from build123d import *

# Parameters (mm, degrees)
SKETCH1_W             = 220
SKETCH1_H             = 90
BOSS_EXTRUDE1_DEPTH   = 15
M6_TAPPED_HOLE1_D     = 5
M6_TAPPED_HOLE1_DEPTH = 15
M6_TAPPED_HOLE1_TIP   = 1.502151548
CUT_EXTRUDE1_DEPTH    = 239.170107276
CUT_EXTRUDE2_DEPTH    = 239.170107276
M6_TAPPED_HOLE2_D     = 5
M6_TAPPED_HOLE2_DEPTH = 15
M6_TAPPED_HOLE2_TIP   = 1.502151548
CHAMFER1_SIZE         = 5
FILLET1_R             = 5
CUT_EXTRUDE3_DEPTH    = 6
SKETCH11_R            = 2.5
CUT_EXTRUDE4_DEPTH    = 239.170107276


with BuildPart() as part:
    # Sketch1 → Boss-Extrude1 (new body)
    with BuildSketch(Plane.XY):
        with Locations((110, 45)):
            Rectangle(SKETCH1_W, SKETCH1_H)
    extrude(amount=BOSS_EXTRUDE1_DEPTH)

    # M6 Tapped Hole1
    with Locations(Plane.XY.offset(15)):
        with Locations((70, 73), (70, 17), (200, 73), (200, 17)):
            Hole(M6_TAPPED_HOLE1_D / 2, depth=M6_TAPPED_HOLE1_DEPTH)
            with Locations((0, 0, -(M6_TAPPED_HOLE1_DEPTH + M6_TAPPED_HOLE1_TIP / 2))):  # 118° drill point
                Cone(0, M6_TAPPED_HOLE1_D / 2, M6_TAPPED_HOLE1_TIP, mode=Mode.SUBTRACT)

    # Sketch4 → Cut-Extrude1 (cut, through all)
    with BuildSketch(Plane.XY.offset(15)):
        with BuildLine():
            Line((44.5, 80), (44.5, 70))
            ThreePointArc((44.5, 70), (40, 65.5), (35.5, 70))
            Line((35.5, 70), (35.5, 80))
            ThreePointArc((35.5, 80), (40, 84.5), (44.5, 80))
        make_face()
        with BuildLine():
            Line((44.5, 20), (44.5, 10))
            ThreePointArc((44.5, 10), (40, 5.5), (35.5, 10))
            Line((35.5, 10), (35.5, 20))
            ThreePointArc((35.5, 20), (40, 24.5), (44.5, 20))
        make_face()
        with BuildLine():
            Line((174.5, 80), (174.5, 70))
            ThreePointArc((174.5, 70), (170, 65.5), (165.5, 70))
            Line((165.5, 70), (165.5, 80))
            ThreePointArc((165.5, 80), (170, 84.5), (174.5, 80))
        make_face()
        with BuildLine():
            Line((174.5, 20), (174.5, 10))
            ThreePointArc((174.5, 10), (170, 5.5), (165.5, 10))
            Line((165.5, 10), (165.5, 20))
            ThreePointArc((165.5, 20), (170, 24.5), (174.5, 20))
        make_face()
    extrude(amount=-CUT_EXTRUDE1_DEPTH, mode=Mode.SUBTRACT)

    # Sketch5 → Cut-Extrude2 (cut, through all)
    with BuildSketch(Plane.XY.offset(15)):
        Polygon((72.318759133, 0), (116.159379566, 43.840620434), (160, 0), (116.159379566, -43.840620434), align=None)
    extrude(amount=-CUT_EXTRUDE2_DEPTH, mode=Mode.SUBTRACT)

    # M6 Tapped Hole2
    with Locations(Plane(origin=(0, 90, 0), x_dir=(1, 0, 0), z_dir=(0, 1, 0))):
        with Locations((80, -9)):
            Hole(M6_TAPPED_HOLE2_D / 2, depth=M6_TAPPED_HOLE2_DEPTH)
            with Locations((0, 0, -(M6_TAPPED_HOLE2_DEPTH + M6_TAPPED_HOLE2_TIP / 2))):  # 118° drill point
                Cone(0, M6_TAPPED_HOLE2_D / 2, M6_TAPPED_HOLE2_TIP, mode=Mode.SUBTRACT)

    # Chamfer1
    chamfer1_edges = [part.edges().sort_by_distance(p)[0] for p in [
        (0, 90, 7.5),
        (220, 90, 7.5),
        (220, 0, 7.5),
        (0, 0, 7.5),
    ]]
    chamfer(chamfer1_edges, length=CHAMFER1_SIZE)

    # Fillet1
    fillet1_edges = [part.edges().sort_by_distance(p)[0] for p in [
        (116.159379566, 43.840620434, 7.5),
    ]]
    fillet(fillet1_edges, radius=FILLET1_R)

    # Sketch10 → Cut-Extrude3 (cut)
    with BuildSketch(Plane(origin=(0, 0, 0), x_dir=(-1, 0, 0), z_dir=(0, 0, -1))):
        with BuildLine():
            Line((-153, 0), (-153, 90))
            ThreePointArc((-153, 90), (-150, 93), (-147, 90))
            Line((-147, 90), (-147, 0))
            ThreePointArc((-147, 0), (-150, -3), (-153, 0))
        make_face()
    extrude(amount=-CUT_EXTRUDE3_DEPTH, mode=Mode.SUBTRACT)

    # Sketch11 → Cut-Extrude4 (cut, through all)
    with BuildSketch(Plane.XY.offset(15)):
        with Locations((10, 55)):
            Circle(SKETCH11_R)
        with Locations((10, 35)):
            Circle(SKETCH11_R)
        with Locations((10, 25)):
            Circle(SKETCH11_R)
        with Locations((10, 65)):
            Circle(SKETCH11_R)
        with Locations((10, 75)):
            Circle(SKETCH11_R)
        with Locations((10, 15)):
            Circle(SKETCH11_R)
    extrude(amount=-CUT_EXTRUDE4_DEPTH, mode=Mode.SUBTRACT)


solid = part.part
The listing builds one solid part. Answer for the finished solid, in the listing's coordinates (mm). A direction names the side the tool comes from. Give positions to 0.01 mm unless a question says otherwise; leave off trailing zeros. Write each loop counter-clockwise with the first axis right and the second up, starting at its lowest first coordinate (ties: lowest second). Pieces come first, ordered by that corner, then holes. Notation, with made-up numbers: (60.5, 46) -> (79.5, 46) arc R25 ccw to (79.5, 75) -> close; hole circle Ø11 at (-7, 32). An arc over 180 degrees is marked (long way). Use a Markdown table: item, result.
(1) For faces 4 (the flat face through (165.5, 75, 8)), 5 (the flat face through (72, 56, 0)), 6 (the cylindrical face through (82, 82.4, 10.5)), determine the directions among +Z, -Z, +X, -X, +Y, -Y from which every point of the face is accessible in a straight line to the end or side of a thin tool.
Return value:
| item | result |
|---|---|
| face 4 | +Z, -Z |
| face 5 | -Z, +X, -X, +Y, -Y |
| face 6 | +Y |
(2) Determine the mould class of faces 1 (the flat face through (153, 48, 3)), 2 (the flat face through (218, 87, 7)), 3 (the flat face through (109, 90, 7)) for opening direction X: released by +X, released by -X, zero draft, split by the parting line, or undercut.
Return value:
| item | result |
|---|---|
| face 1 | undercut |
| face 2 | released by +X |
| face 3 | zero draft |
(3) Section C-C, the plane x = 170.5 is taken. Determine the outline of the cut face in (y, z), then the cut area to 3 significant figures.
Return value:
| item | result |
|---|---|
| outline | (0, 0) -> (5.53, 0) -> (5.53, 15) -> (0, 15) -> close; (24.47, 0) -> (65.53, 0) -> (65.53, 15) -> (24.47, 15) -> close; (84.47, 0) -> (90, 0) -> (90, 15) -> (84.47, 15) -> close |
| area | 782 mm2 |
(4) Section A-A, the plane x = 200 is taken. Determine the outline of the cut face in (y, z).
Return value:
| item | result |
|---|---|
| outline | (0, 0) -> (14.5, 0) -> (14.5, 15) -> (0, 15) -> close; (19.5, 0) -> (70.5, 0) -> (70.5, 15) -> (19.5, 15) -> close; (75.5, 0) -> (90, 0) -> (90, 15) -> (75.5, 15) -> close |
(5) Find the intervals of material crossed by probe 1 along Y at (x, z) = (200, 9.5); probe 2 along X at (y, z) = (50.5, 5); probe 3 along X at (y, z) = (79, 10.25), in increasing order. Write a range as from..to.
Return value:
| item | result |
|---|---|
| probe 1 | 0..14.5, 19.5..70.5, 75.5..90 |
| probe 2 | 0..147, 153..220 |
| probe 3 | 0..35.5, 44.5..77.83, 82.17..165.5, 174.5..220 |
(6) Section B-B, the plane y = 55 is taken. Determine the outline of the cut face in (x, z).
Return value:
| item | result |
|---|---|
| outline | (0, 0) -> (7.5, 0) -> (7.5, 15) -> (0, 15) -> close; (12.5, 0) -> (147, 0) -> (147, 6) -> (153, 6) -> (153, 0) -> (220, 0) -> (220, 15) -> (12.5, 15) -> close |
(7) A flat-ended cylindrical pin translates along its axis: P1, Ø6, axis at x = 80, z = 9, coming from the +Y side. Find the tip coordinate at first contact, or state that the pin passes through.
Return value:
| item | result |
|---|---|
| P1 | y = 90 |
